from build123d import *

# Parameters (mm, degrees)
BOLT_ROD_SWEEP_7_5_PROFILE_R = 3.75


with BuildPart() as part:
    # Bolt Rod Sweep Ø7.5: sweep along a path in Bolt Rod Path
    with BuildLine(Plane.XY) as bolt_rod_sweep_7_5_path:
        Line((0, 0), (0, -25))
        ThreePointArc((0, -25), (-1.464466094, -28.535533906), (-5, -30))
        Line((-5, -30), (-63.25, -30))
        ThreePointArc((-63.25, -30), (-66.785533906, -28.535533906), (-68.25, -25))
        Line((-68.25, -25), (-68.25, 5))
        ThreePointArc((-68.25, 5), (-66.785533906, 8.535533906), (-63.25, 10))
        Line((-63.25, 10), (73.75, 10))
    # Bolt Rod Sweep Ø7.5 profile (on start of the path) → Bolt Rod Sweep Ø7.5 (sweep)
    with BuildSketch(Plane(origin=(0, 0, 0), x_dir=(-1, 0, 0), z_dir=(0, -1, 0))):
        Circle(BOLT_ROD_SWEEP_7_5_PROFILE_R)
    sweep(path=bolt_rod_sweep_7_5_path.line)


solid = part.part
The listing builds one solid part. Answer for the finished solid, in the listing's coordinates (mm). A direction names the side the tool comes from. Give positions to 0.01 mm unless a question says otherwise; leave off trailing zeros. Order: outer loops, then holes, each group sorted by start corner. A loop starts at its lowest first (then second) coordinate and runs counter-clockwise, first axis right, second up. Notation, with made-up numbers: (-17, 53) - (-5, 53) arc R27 ccw to (-5, 76) - close; hole circle Ø9 at (8.25, -32). An arc over 180 degrees is marked (long way). Use one line per item in the form item = value.
1) Find section B-B on z = 0. Determine the outline of the cut face in (x, y), and give its area (3 significant figures).
Verdict:
outline = (-72, -25) arc R8.75 ccw to (-63.25, -33.75) - (-5, -33.75) arc R8.75 ccw to (3.75, -25) - (3.75, 0) - (-3.75, 0) - (-3.75, -25) arc R1.25 cw to (-5, -26.25) - (-63.25, -26.25) arc R1.25 cw to (-64.5, -25) - (-64.5, 5) arc R1.25 cw to (-63.25, 6.25) - (73.75, 6.25) - (73.75, 13.75) - (-63.25, 13.75) arc R8.75 ccw to (-72, 5) - close
area = 2,050 mm^2
2) Find section D-D on x = 59. Determine the outline of the cut face in (y, z), and give its area (3 significant figures).
Verdict:
outline = circle Ø7.5 at (10, 0)
area = 44.2 mm^2
3) The mould has two halves that part along Y. Classify faces 1 (the flat face through (73.75, 10, 0)), 2 (the flat face through (0, 0, 0)): released by +Y, released by -Y, zero draft, split by the parting line, or undercut.
Verdict:
face_1 = zero draft
face_2 = undercut
4) Find section A-A on y = -17. Determine the outline of the cut face in (x, z).
Verdict:
outline = circle Ø7.5 at (-68.25, 0); circle Ø7.5 at (0, 0)
5) Find section C-C on x = -18. Determine the outline of the cut face in (y, z), and give its area (3 significant figures).
Verdict:
outline = circle Ø7.5 at (-30, 0); circle Ø7.5 at (10, 0)
area = 88.4 mm^2
6) Consider probe 1 along Y at (x, z) = (-32, -0.25); probe 2 along X at (y, z) = (-9, 0); probe 3 along Y at (x, z) = (-47.5, 1.75). Determine where each line is inside the solid, lowest interval first. Write a range as [from, to].
Verdict:
probe_1 = [-33.74, -26.26], [6.26, 13.74]
probe_2 = [-72, -64.5], [-3.75, 3.75]
probe_3 = [-33.32, -26.68], [6.68, 13.32]
7) For faces 3 (the cylindrical face through (-34.533, -33.746, -0.165)), 4 (the cylindrical face through (6.209, 13.746, -0.165)), determine the directions among +Z, -Z, +X, -X, +Y, -Y from which every point of the face is accessible in a straight line to the end or side of a thin tool.
Verdict:
face_3 = none
face_4 = +X
8) Each of these flat-tipped pins is pushed along its axis until it touches: pin 1 (3 mm diameter, centred on x = 33, y = 4, fed in from -Z); pin 2 (1 mm diameter, centred on x = 18.5, z = -0.5, fed in from -Y). Where does it stop, or does it pass through?
Verdict:
pin_1 = through
pin_2 = 6.25
